from build123d import *

# Parameters (mm, degrees)
SIDE_ARM_16MM_DEPTH          = 16
BRACKET_BODY_94MM_DEPTH      = 94
SECOND_START                 = -16
SECOND_ARM_16MM_DEPTH        = 16
PIVOT_HOLE_SKETCH_14_R       = 7
PIVOT_HOLES_14_THROUGH_DEPTH = 231
BEARING_BOSS_45_DEPTH        = 8
BEARING_BOSS_45_DEPTH_BACK   = 12
BEARING_BOSS_SKETCH_45_R     = 22.5
BOSS_SUPPORT_WEB_12MM_DEPTH  = 12
BEARING_BORE_SKETCH_20_R     = 10
BEARING_BORE_20_DEPTH        = 101
COUNTERBORE_SKETCH_24_R      = 12
COUNTERBORES_24X6_DEPTH      = 6
MOUNTING_HOLE_SKETCH_12_R    = 6
MOUNTING_HOLES_12_DEPTH      = 58


with BuildPart() as part:
    # Side Arm Profile → Side Arm 16mm (new body)
    with BuildSketch(Plane(origin=(0, 0, 0), x_dir=(0, 0, -1), z_dir=(1, 0, 0))):
        with BuildLine():
            Line((0, 0), (-20, 0))
            Line((-20, 0), (-20, 20))
            Line((-20, 20), (-40, 20))
            Line((-40, 20), (-40, 0))
            Line((-40, 0), (-96, 0))
            ThreePointArc((-96, 0), (-109.516186166, 10.351341133), (-103.045136072, 26.098184068))
            Line((-103.045136072, 26.098184068), (-62, 50))
            Line((-62, 50), (-50, 50))
            Line((-50, 50), (-50, 35))
            Line((-50, 35), (0, 35))
            Line((0, 35), (0, 0))
        make_face()
    extrude(amount=-SIDE_ARM_16MM_DEPTH)

    # Bracket Body Profile → Bracket Body 94mm (add)
    with BuildSketch(Plane.ZY.offset(16)):
        Polygon((0, 0), (0, 35), (50, 35), (50, 50), (62, 50), (62, 0), (40, 0), (40, 20), (20, 20), (20, 0), align=None)
    extrude(amount=BRACKET_BODY_94MM_DEPTH)

    # Second Arm Profile → Second Arm 16mm (add)
    with BuildSketch(Plane.ZY.offset(110).offset(SECOND_START)):
        with BuildLine():
            Line((62, 0), (62, 50))
            Line((62, 50), (103.045136072, 26.098184068))
            ThreePointArc((103.045136072, 26.098184068), (109.516186166, 10.351341133), (96, 0))
            Line((96, 0), (62, 0))
        make_face()
    extrude(amount=SECOND_ARM_16MM_DEPTH)

    # Pivot Hole Sketch Ø14 → Pivot Holes Ø14 Through (cut)
    with BuildSketch(Plane(origin=(0, 0, 0), x_dir=(0, 0, -1), z_dir=(1, 0, 0))):
        with Locations((-96, 14)):
            Circle(PIVOT_HOLE_SKETCH_14_R)
    extrude(amount=-PIVOT_HOLES_14_THROUGH_DEPTH, mode=Mode.SUBTRACT)



with BuildPart() as body_2:
    # Bearing Boss Sketch Ø45 → Bearing Boss Ø45 (new, two sides: drawn at the far end of the back side and taken through both)
    with BuildSketch(Plane.XY.offset(62).offset(-BEARING_BOSS_45_DEPTH_BACK)):
        with Locations((-47, 83)):
            Circle(BEARING_BOSS_SKETCH_45_R)
    extrude(amount=BEARING_BOSS_45_DEPTH + BEARING_BOSS_45_DEPTH_BACK)


with BuildPart() as part_1:
    add(part.part)

    add(body_2.part)  # Boss Support Web 12mm merges body 2
    # Boss Support Web Profile → Boss Support Web 12mm (add)
    with BuildSketch(Plane.XY.offset(62)):
        with BuildLine():
            Line((-20, 50), (-24.5, 83))
            ThreePointArc((-24.5, 83), (-47, 60.5), (-69.5, 83))
            Line((-69.5, 83), (-74, 50))
            Line((-74, 50), (-20, 50))
        make_face()
    extrude(amount=-BOSS_SUPPORT_WEB_12MM_DEPTH)

    # Bearing Bore Sketch Ø20 → Bearing Bore Ø20 (cut)
    with BuildSketch(Plane.XY.offset(70)):
        with Locations((-47, 83)):
            Circle(BEARING_BORE_SKETCH_20_R)
    extrude(amount=-BEARING_BORE_20_DEPTH, mode=Mode.SUBTRACT)

    # Counterbore Sketch Ø24 → Counterbores Ø24x6 (cut)
    with BuildSketch(Plane(origin=(0, 35, 0), x_dir=(1, 0, 0), z_dir=(0, 1, 0))):
        with Locations(Location((-20, -20, 0), (0, 0, 270))):
            Circle(COUNTERBORE_SKETCH_24_R)
        with Locations(Location((-55, -20, 0), (0, 0, 270))):
            Circle(COUNTERBORE_SKETCH_24_R)
        with Locations(Location((-90, -20, 0), (0, 0, 270))):
            Circle(COUNTERBORE_SKETCH_24_R)
    extrude(amount=-COUNTERBORES_24X6_DEPTH, mode=Mode.SUBTRACT)

    # Mounting Hole Sketch Ø12 → Mounting Holes Ø12 (cut)
    with BuildSketch(Plane(origin=(0, 29, 0), x_dir=(1, 0, 0), z_dir=(0, 1, 0))):
        with Locations(Location((-20, -20, 0), (0, 0, 270))):
            Circle(MOUNTING_HOLE_SKETCH_12_R)
        with Locations(Location((-55, -20, 0), (0, 0, 270))):
            Circle(MOUNTING_HOLE_SKETCH_12_R)
        with Locations(Location((-90, -20, 0), (0, 0, 270))):
            Circle(MOUNTING_HOLE_SKETCH_12_R)
    extrude(amount=-MOUNTING_HOLES_12_DEPTH, mode=Mode.SUBTRACT)


solid = part_1.part
Design review of the part built by this model. Coordinates are the model's own, in mm. A direction names the side the tool comes from. Round coordinates to 2 decimals unless told otherwise and drop trailing zeros. Write each loop counter-clockwise with the first axis right and the second up, starting at its lowest first coordinate (ties: lowest second). Pieces come first, ordered by that corner, then holes. Notation, with made-up numbers: (24, -18.75) -> (59, -18.75) arc R17 ccw to (59, -2.75) -> close; hole circle Ø5 at (64.5, 18). An arc over 180 degrees is marked (long way). One line per item, written item: value. Start each with the question number.
Q1. Add section A-A (y = 14). Give the boundary of the cut face in (x, z), then the cut area to 3 significant figures.
Q2. Add section C-C (y = 78). Give the boundary of the cut face in (x, z), then the cut area to 3 significant figures.
Q3. Add section B-B (x = -90). Give the boundary of the cut face in (y, z).
Q4. Tool access review of faces 4 (the face through (-66.715, 32.042, 17.399)), 5 (the face through (-56, 63, 50)), 6 (the face through (-92, 50, 56)): name each direction out of +Z, -Z, +X, -X, +Y, -Y from which nothing blocks a thin tool from reaching the whole face with its end or side.
Q5. The part is to be moulded in two halves that separate along X. For faces 1 (the face through (-54, 0, 56)), 2 (the face through (-94, 20, 81)), 3 (the face through (-110, 20, 56)), say which applies: pulls with the +X half, pulls with the -X half, needs draft (parallel to the pull), parting line crosses it, or undercut.
Q6. To check wall thickness, follow probe 1 along X at (y, z) = (28, 68); probe 2 along Z at (x, y) = (-20, 15); probe 3 along Z at (x, y) = (-37, 14.5). State the ranges of each line that lie inside material, in increasing order.
Q7. Add section D-D (x = -55). Give the boundary of the cut face in (y, z).
Q8. Insertion check: P1, Ø6, axis at x = -14, z = 55.5, coming from the +Y side; P2, Ø10, axis at x = -49, z = 26.5, coming from the +Y side; P3, Ø6, axis at x = -61, z = 32, coming from the -Y side; P4, Ø8.5, axis at y = 14, z = 96, coming from the +X side. Each pin has a flat end and moves straight along its axis. Give the tip position at first contact, or say it passes through.
Response:
1. outline: (-110, 0) -> (0, 0) -> (0, 20) -> (-14, 20) arc R6 cw to (-26, 20) -> (-49, 20) arc R6 cw to (-61, 20) -> (-84, 20) arc R6 cw to (-96, 20) -> (-110, 20) -> close; (-110, 40) -> (0, 40) -> (0, 89) -> (-16, 89) -> (-16, 62) -> (-94, 62) -> (-94, 89) -> (-110, 89) -> close; (-110, 103) -> (-94, 103) -> (-94, 110) -> (-110, 110) -> close; (-16, 103) -> (0, 103) -> (0, 110) -> (-16, 110) -> close
1. area: 5,540 mm^2
2. outline: (-70.18, 50) -> (-55.66, 50) -> (-55.66, 70) -> (-68.94, 70) -> (-68.94, 62) -> (-70.18, 62) -> close; (-38.34, 50) -> (-23.82, 50) -> (-23.82, 62) -> (-25.06, 62) -> (-25.06, 70) -> (-38.34, 70) -> close
2. area: 561 mm^2
3. outline: (0, 0) -> (35, 0) -> (35, 8) -> (29, 8) -> (29, 14) -> (0, 14) -> close; (0, 40) -> (20, 40) -> (20, 26) -> (29, 26) -> (29, 32) -> (35, 32) -> (35, 50) -> (50, 50) -> (50, 62) -> (0, 62) -> close
4. face 4: +Y
4. face 5: -Z, +X, -X, +Y
4. face 6: +Z, -Z, -X, +Y
5. face 1: needs draft
5. face 2: undercut
5. face 3: pulls with the -X half
6. probe 1: x = -110 to -94, -16 to 0
6. probe 2: z = 0 to 14, 40 to 62
6. probe 3: z = 0 to 20, 40 to 62
7. outline: (0, 0) -> (35, 0) -> (35, 8) -> (29, 8) -> (29, 14) -> (0, 14) -> close; (0, 40) -> (20, 40) -> (20, 26) -> (29, 26) -> (29, 32) -> (35, 32) -> (35, 50) -> (77, 50) -> (77, 70) -> (61.97, 70) -> (61.97, 62) -> (0, 62) -> close; (89, 50) -> (104.03, 50) -> (104.03, 70) -> (89, 70) -> close
8. P1: stops at y = 50
8. P2: stops at y = 35
8. P3: stops at y = 20
8. P4: passes through
